Geometry: final body of the model. Coordinates: model frame, mm. Face numbers are marked on the shaded views. Give positions to 0.01 mm unless a question says otherwise; leave off trailing zeros. Loops run counter-clockwise (first coordinate to the right, second up) from the corner with the lowest first, then second, coordinate; pieces in that order, holes last.
1. Section C-C, the plane z = 3. Output: boundary loops of the cut face in (x, y).
2. Section B-B, the plane x = 0. Output: boundary loops of the cut face in (y, z).
3. Section D-D, the plane x = -19. Output: boundary loops of the cut face in (y, z).
4. Draft query along Y for the marked faces 1, 2 and 3. Return one class per face: +Y half, -Y half, draft (parallel to the pull), parting line (faces both ways), or undercut.
5. Material intervals for line 1 along Y through (x, z) = (0, 2.75); line 2 along X through (y, z) = (56.5, 2); line 3 along Y through (x, z) = (34, 6), sorted ascending.
6. First-contact query: P1, Ø3, axis at y = -36, z = 9.5, coming from the +X side; P2, Ø2, axis at x = 15.5, z = 3, coming from the -Y side (3 decimals); P3, Ø8, axis at x = 44, z = 2, coming from the -Y side. Flat tips, straight axial feed; report the tip coordinate or a pass-through.
7. Section A-A, the plane y = 0. Output: boundary loops of the cut face in (x, z), then the cut area to 3 significant figures.
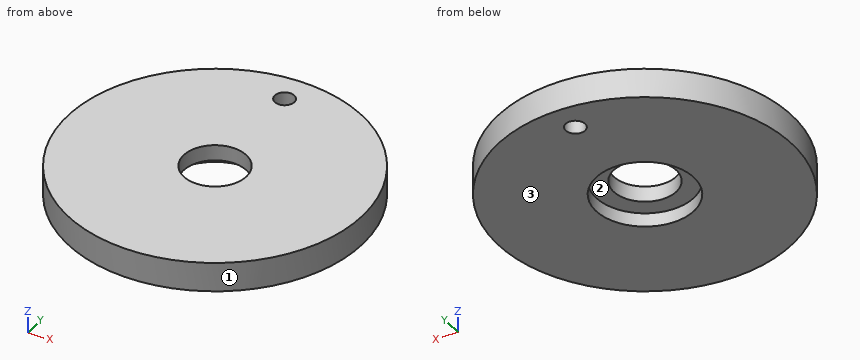
from build123d import *

# Parameters (mm, degrees)
SKETCH_1_R          = 75
SKETCH_1_R_2        = 5
SKETCH_1_R_3        = 16
EXTRUDE_1_DEPTH     = 15
CUT_EXTRUDE_START   = -15
SKETCH_2_R          = 25
CUT_EXTRUDE_1_DEPTH = 7


with BuildPart() as part:
    # 草图1 → 凸台-拉伸1 (new body)
    with BuildSketch(Plane.XY):
        Circle(SKETCH_1_R)
        with Locations((0, 60)):
            Circle(SKETCH_1_R_2, mode=Mode.SUBTRACT)
        Circle(SKETCH_1_R_3, mode=Mode.SUBTRACT)
    extrude(amount=EXTRUDE_1_DEPTH)

    # 草图2 → 切除-拉伸1 (cut)
    with BuildSketch(Plane.XY.offset(15).offset(CUT_EXTRUDE_START)):
        Circle(SKETCH_2_R)
    extrude(amount=CUT_EXTRUDE_1_DEPTH, mode=Mode.SUBTRACT)


solid = part.part
Answers below:
1. outline: circle Ø150 at (0, 0); hole circle Ø50 at (0, 0); hole circle Ø10 at (0, 60)
2. outline: (-75, 0) - (-25, 0) - (-25, 7) - (-16, 7) - (-16, 15) - (-75, 15) - close; (16, 7) - (25, 7) - (25, 0) - (55, 0) - (55, 15) - (16, 15) - close; (65, 0) - (75, 0) - (75, 15) - (65, 15) - close
3. outline: (-72.55, 0) - (-16.25, 0) - (-16.25, 7) - (16.25, 7) - (16.25, 0) - (72.55, 0) - (72.55, 15) - (-72.55, 15) - close
4. face 1: parting line
4. face 2: undercut
4. face 3: draft
5. line 1: y = -75 to -25, 25 to 55, 65 to 75
5. line 2: x = -49.32 to -3.57, 3.57 to 49.32
5. line 3: y = -66.85 to 66.85
6. P1: stops at x = 66.59
6. P2: stops at y = -73.585
6. P3: stops at y = -63.44
7. outline: (-75, 0) - (-25, 0) - (-25, 7) - (-16, 7) - (-16, 15) - (-75, 15) - close; (16, 7) - (25, 7) - (25, 0) - (75, 0) - (75, 15) - (16, 15) - close
7. area: 1,640 mm2
